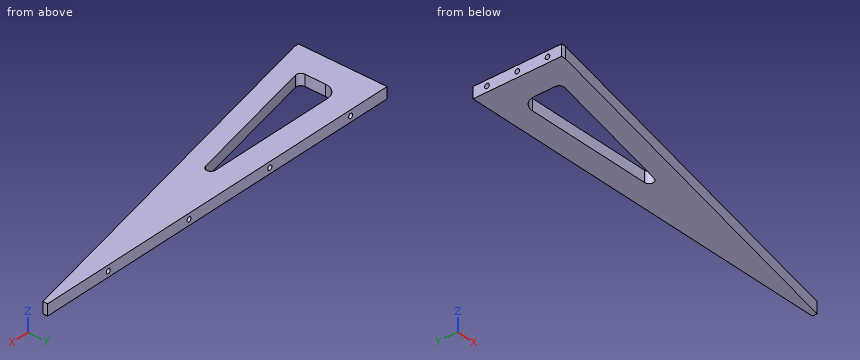
```python
from build123d import *

# Parameters (mm, degrees)
BOSS_EXTRUDE1_DEPTH   = 12
M6_TAPPED_HOLE1_D     = 5
M6_TAPPED_HOLE1_DEPTH = 15
M6_TAPPED_HOLE1_TIP   = 1.502151548
M6_TAPPED_HOLE2_D     = 5
M6_TAPPED_HOLE2_DEPTH = 15
M6_TAPPED_HOLE2_TIP   = 1.502151548


with BuildPart() as part:
    # Sketch1 → Boss-Extrude1 (new body)
    with BuildSketch(Plane.XY):
        Polygon((0, -95), (0, 0), (420, 0), (420, -5), (5, -95), align=None)
        with BuildLine():
            Line((30, -62.172928769), (30, -40))
            ThreePointArc((30, -40), (34.393398282, -29.393398282), (45, -25))
            Line((45, -25), (183.352949325, -25))
            ThreePointArc((183.352949325, -25), (188.324471362, -29.467112929), (184.412653251, -34.886412548))
            Line((184.412653251, -34.886412548), (36.059703926, -67.059341317))
            ThreePointArc((36.059703926, -67.059341317), (31.861411116, -66.065133776), (30, -62.172928769))
        make_face(mode=Mode.SUBTRACT)
    extrude(amount=BOSS_EXTRUDE1_DEPTH)

    # M6 Tapped Hole1
    with Locations(Plane.ZY):
        with Locations((6, -15), (6, -47.5), (6, -80)):
            Hole(M6_TAPPED_HOLE1_D / 2, depth=M6_TAPPED_HOLE1_DEPTH)
            with Locations((0, 0, -(M6_TAPPED_HOLE1_DEPTH + M6_TAPPED_HOLE1_TIP / 2))):  # 118° drill point
                Cone(0, M6_TAPPED_HOLE1_D / 2, M6_TAPPED_HOLE1_TIP, mode=Mode.SUBTRACT)

    # M6 Tapped Hole2
    with Locations(Plane(origin=(0, 0, 0), x_dir=(-1, 0, 0), z_dir=(0, 1, 0))):
        with Locations((-45, 6), (-145, 6), (-245, 6), (-345, 6)):
            Hole(M6_TAPPED_HOLE2_D / 2, depth=M6_TAPPED_HOLE2_DEPTH)
            with Locations((0, 0, -(M6_TAPPED_HOLE2_DEPTH + M6_TAPPED_HOLE2_TIP / 2))):  # 118° drill point
                Cone(0, M6_TAPPED_HOLE2_D / 2, M6_TAPPED_HOLE2_TIP, mode=Mode.SUBTRACT)


solid = part.part
```
CAD build for the part. Positions are in the model's coordinates, mm. Coordinates: 2 decimals unless noted, no trailing zeros. Order: outer loops, then holes, each group sorted by start corner. A loop starts at its lowest first (then second) coordinate and runs counter-clockwise, first axis right, second up. Notation, with made-up numbers: (27, 86) -> (80, 86) arc R27 cw to (80, 117) -> close; hole circle Ø10 at (-7.5, 15.25). An arc over 180 degrees is marked (long way). Use one line per item in the form item = value. Start each with the question number.
1) Band-saw the part on B-B on x = 133.5. Give the cut face in (y, z), then the cut area to 3 significant figures.
2) Drop flat-ended pins along their axis: pin 1 (3 mm diameter, centred on x = 245, z = 6, fed in from +Y); pin 2 (4 mm diameter, centred on x = 345, z = 6, fed in from -Y). Give the stop position or say it passes through.
3) Drill centre lines: L1, parallel to Z at x = 145, y = -11.25; L2, parallel to Y at x = 8.5, z = 6; L3, parallel to Y at x = 11, z = 6. Where is each one in solid material? Low to high. Write a range as [from, to].
4) Band-saw the part on A-A on y = -58.5. Give the cut face in (x, z), then the cut area to 3 significant figures.
5) Band-saw the part on C-C on x = 282. Give the cut face in (y, z), then the cut area to 3 significant figures.
Entries:
q1.outline = (-67.13, 0) -> (-45.93, 0) -> (-45.93, 12) -> (-67.13, 12) -> close; (-25, 0) -> (0, 0) -> (0, 12) -> (-25, 12) -> close
q1.area = 554 mm2
q2.pin_1 = -15.6
q2.pin_2 = -21.7
q3.L1 = [0, 3.5], [8.5, 12]
q3.L2 = [-94.24, -82.5], [-77.5, -50], [-45, -17.5], [-12.5, 0]
q3.L3 = [-93.7, -82.5], [-77.5, -50], [-45, -17.5], [-12.5, 0]
q4.outline = (0, 0) -> (30, 0) -> (30, 12) -> (0, 12) -> close; (75.53, 0) -> (173.31, 0) -> (173.31, 12) -> (75.53, 12) -> close
q4.area = 1,530 mm2
q5.outline = (-34.93, 0) -> (0, 0) -> (0, 12) -> (-34.93, 12) -> close
q5.area = 419 mm2
